Work out the finished part from the listing and answer in its coordinate system (mm). A direction names the side the tool comes from. Coordinates: 2 decimals unless noted, no trailing zeros. Order: outer loops, then holes, each group sorted by start corner. A loop starts at its lowest first (then second) coordinate and runs counter-clockwise, first axis right, second up. Notation, with made-up numbers: M 5.5,60.5 L 10.5,60.5 A18 ccw 10.5,77.5 Z; hole C -13,2.25 d5. An arc over 180 degrees is marked long. Write item = value, one per line. Start each with the question number.
Q1. Each of these flat-tipped pins is pushed along its axis until it touches: P1, Ø1.2, axis at x = -8, y = 2.5, coming from the +Z side; P2, Ø1.2, axis at x = -10.5, y = 2.5, coming from the -Z side. Where does it stop, or does it pass through?
Q2. Find section B-B on y = 3.05. Give the vertices of the cut face in (x, z).
Q3. Straight lines are drawn through the part: line 1 along X through (y, z) = (2.5, 0); line 2 along Z through (x, y) = (-15, 2.6); line 3 along Z through (x, y) = (-7, 0.8). For each, find the intervals that lie inside material, in ascending order.
Q4. A tool of negligible diameter and unlimited length cuts with its end or side. For faces 1 (the cylindrical face through (17, 2, 0)), 2 (the flat face through (-10, 2, 3.5)), 3 (the flat face through (10, 2, 3.5)), 4 (the flat face through (10, 2, -3.5)), from which of +Z, -Z, +X, -X, +Y, -Y can it reach the whole face along a straight path? Write none if from no direction.
Q5. Find section D-D on z = -1.5. Give the vertices of the cut face in (x, y), and give its area (3 significant figures).
Q6. Find section A-A on z = 0. Give the vertices of the cut face in (x, y).
Q7. Determine the mould class of faces 5 (the cylindrical face through (0, 2, -5)), 6 (the cylindrical face through (3.7, 2, -3.6)), 7 (the flat face through (-10, 2, -3.5)), 8 (the cylindrical face through (-17, 2, 0)) for opening direction X: released by +X, released by -X, zero draft, split by the parting line, or undercut.
Q8. Find section C-C on x = 0. Give the vertices of the cut face in (y, z), and give its area (3 significant figures).
```python
from build123d import *

# Parameters (mm, degrees)
SKETCH1_R           = 5
SKETCH1_R_2         = 4
BOSS_EXTRUDE1_DEPTH = 8
SCALE1_SCALE        = 0.5


with BuildPart() as part:
    # Sketch1 → Boss-Extrude1 (new body)
    with BuildSketch(Plane(origin=(0, 0, 0), x_dir=(1, 0, 0), z_dir=(0, 1, 0))):
        with BuildLine():
            Line((30, 7), (8.660254038, 7))
            ThreePointArc((8.660254038, 7), (7.350946696, 7.22035527), (6.185895741, 7.857142857))
            ThreePointArc((6.185895741, 7.857142857), (0, 10), (-6.185895741, 7.857142857))
            ThreePointArc((-6.185895741, 7.857142857), (-7.350946696, 7.22035527), (-8.660254038, 7))
            Line((-8.660254038, 7), (-30, 7))
            ThreePointArc((-30, 7), (-37, 0), (-30, -7))
            Line((-30, -7), (-8.660254038, -7))
            ThreePointArc((-8.660254038, -7), (-7.350946696, -7.22035527), (-6.185895741, -7.857142857))
            ThreePointArc((-6.185895741, -7.857142857), (0, -10), (6.185895741, -7.857142857))
            ThreePointArc((6.185895741, -7.857142857), (7.350946696, -7.22035527), (8.660254038, -7))
            Line((8.660254038, -7), (30, -7))
            ThreePointArc((30, -7), (37, 0), (30, 7))
        make_face()
        with Locations(Location((0, 0, 0), (0, 0, 270))):
            Circle(SKETCH1_R, mode=Mode.SUBTRACT)
        with Locations(Location((30, 0, 0), (0, 0, 270))):
            Circle(SKETCH1_R_2, mode=Mode.SUBTRACT)
        with Locations(Location((-30, 0, 0), (0, 0, 90))):
            Circle(SKETCH1_R_2, mode=Mode.SUBTRACT)
    extrude(amount=BOSS_EXTRUDE1_DEPTH)


with BuildPart() as part_1:
    # Scale1: scaled about (0, 0, 0)
    add(part.part.scale(SCALE1_SCALE))


solid = part_1.part
```
Findings below:
q1.P1 = 3.5
q1.P2 = -3.5
q2.outline = M -15,-3.5 L -4.33,-3.5 A2 cw -3.09,-3.93 A5 ccw 3.09,-3.93 A2 cw 4.33,-3.5 L 15,-3.5 A3.5 ccw 15,3.5 L 4.33,3.5 A2 cw 3.09,3.93 A5 ccw -3.09,3.93 A2 cw -4.33,3.5 L -15,3.5 A3.5 ccw Z; hole C -15,0 d4; hole C 0,0 d5; hole C 15,0 d4
q3.line_1 = -18.5 to -17, -13 to -2.5, 2.5 to 13, 17 to 18.5
q3.line_2 = -3.5 to -2, 2 to 3.5
q3.line_3 = -3.5 to 3.5
q4.face_1 = +Y, -Y
q4.face_2 = +Z, -X, +Y, -Y
q4.face_3 = +Z, +X, +Y, -Y
q4.face_4 = -Z, +X, +Y, -Y
q5.outline = M -18.16,0 L -16.32,0 L -16.32,4 L -18.16,4 Z; M -13.68,0 L -2,0 L -2,4 L -13.68,4 Z; M 2,0 L 13.68,0 L 13.68,4 L 2,4 Z; M 16.32,0 L 18.16,0 L 18.16,4 L 16.32,4 Z
q5.area = 108 mm^2
q6.outline = M -18.5,0 L -17,0 L -17,4 L -18.5,4 Z; M -13,0 L -2.5,0 L -2.5,4 L -13,4 Z; M 2.5,0 L 13,0 L 13,4 L 2.5,4 Z; M 17,0 L 18.5,0 L 18.5,4 L 17,4 Z
q7.face_5 = split by the parting line
q7.face_6 = released by +X
q7.face_7 = zero draft
q7.face_8 = undercut
q8.outline = M 0,-5 L 4,-5 L 4,-2.5 L 0,-2.5 Z; M 0,2.5 L 4,2.5 L 4,5 L 0,5 Z
q8.area = 20.0 mm^2
